For this review, take the finished solid that the model builds, in its own axes (mm). Coordinates: 2 decimals unless noted, no trailing zeros. Write each loop counter-clockwise with the first axis right and the second up, starting at its lowest first coordinate (ties: lowest second). Pieces come first, ordered by that corner, then holes. Notation, with made-up numbers: M -34.75,38.25 L -27.75,38.25 A36 cw -27.75,77.25 Z; hole C -29.5,29 d1. An arc over 180 degrees is marked long. Return JSON: item names as keys, results as strings.
```python
from build123d import *

# Parameters (mm, degrees)
SKETCH1_R           = 26.2509
SKETCH1_R_2         = 4.5
BOSS_EXTRUDE1_DEPTH = 9.525


with BuildPart() as part:
    # Sketch1 → Boss-Extrude1 (new body)
    with BuildSketch(Plane.XY.offset(222.25)):
        with BuildLine():
            Line((-8.950572213, 93.257741865), (-24.018992106, 51.857598462))
            ThreePointArc((-24.018992106, 51.857598462), (0, -57.15), (24.018992106, 51.857598462))
            Line((24.018992106, 51.857598462), (8.950572213, 93.257741865))
            ThreePointArc((8.950572213, 93.257741865), (0, 99.525), (-8.950572213, 93.257741865))
        make_face()
        with Locations(Location((0, 0, 0), (0, 0, 180))):
            Circle(SKETCH1_R, mode=Mode.SUBTRACT)
        with Locations(Location((0, 90, 0), (0, 0, 180))):
            Circle(SKETCH1_R_2, mode=Mode.SUBTRACT)
    extrude(amount=BOSS_EXTRUDE1_DEPTH)


solid = part.part
```
1. Clearance check with flat-ended pins moving along their axes: pin 1 Ø3 at (x, z) = (-4.5, 223) entering from -Y; pin 2 Ø4 at (y, z) = (-30.5, 223.5) entering from +X; pin 3 Ø1.5 at (y, z) = (38, 225.5) entering from -X; pin 4 Ø14.5 at (x, y) = (0, 90) entering from +Z (3 decimals). State where each tip first meets the part, or that it passes through.
Checks:
{"pin 1": "y = -57.07", "pin 2": "x = 49.54", "pin 3": "x = -43.34", "pin 4": "z = 231.775"}
2. We need section D-D (x = 15). State the section outline as (y, z) points (3 decimals).
Checks:
{"outline": "M -55.146,222.25 L -21.543,222.25 L -21.543,231.775 L -55.146,231.775 Z; M 21.543,222.25 L 76.637,222.25 L 76.637,231.775 L 21.543,231.775 Z"}
3. Draft analysis for pull direction X (two halves, no side actions). For faces 1 (the face through (3.417, -26.028, 226.946)), 2 (the face through (16.59, 72.27, 226.95)), 3 (the face through (-26, 5, 231.775)), 4 (the face through (0.59, 85.54, 226.95)), state which applies: +X half, -X half, draft (parallel to the pull), parting line (faces both ways), or undercut.
Checks:
{"face 1": "undercut", "face 2": "+X half", "face 3": "draft", "face 4": "undercut"}
4. Wall thickness on L1, parallel to X at y = -1, z = 230.5; L2, parallel to Y at x = 4, z = 230.5; L3, parallel to X at y = 90, z = 229: over which ranges is each line inside the solid? List them lowest first. Write a range as from..to.
Checks:
{"L1": "-57.14..-26.23, 26.23..57.14", "L2": "-57.01..-25.94, 25.94..87.94, 92.06..98.64", "L3": "-10.14..-4.5, 4.5..10.14"}
5. We need section B-B (x = 0). State the section outline as (y, z) points (3 decimals), plus the area to 3 significant figures.
Checks:
{"outline": "M -57.15,222.25 L -26.251,222.25 L -26.251,231.775 L -57.15,231.775 Z; M 26.251,222.25 L 85.5,222.25 L 85.5,231.775 L 26.251,231.775 Z; M 94.5,222.25 L 99.525,222.25 L 99.525,231.775 L 94.5,231.775 Z", "area": "907 mm2"}
6. We need section A-A (z = 228). State the section outline as (x, y) points (3 decimals).
Checks:
{"outline": "M -24.019,51.858 A57.15 ccw long 24.019,51.858 L 8.951,93.258 A9.525 ccw -8.951,93.258 Z; hole C 0,0 d52.502; hole C 0,90 d9"}
7. We need section C-C (y = 0). State the section outline as (x, z) points (3 decimals), plus the area to 3 significant figures.
Checks:
{"outline": "M -57.15,222.25 L -26.251,222.25 L -26.251,231.775 L -57.15,231.775 Z; M 26.251,222.25 L 57.15,222.25 L 57.15,231.775 L 26.251,231.775 Z", "area": "589 mm2"}
